Drawing for the job (mm, zero at the part's lowest x, y, z). A direction names the side the tool comes from. Round coordinates to 2 decimals unless told otherwise and drop trailing zeros. Write each loop counter-clockwise with the first axis right and the second up, starting at its lowest first coordinate (ties: lowest second). Pieces come first, ordered by that corner, then holes.
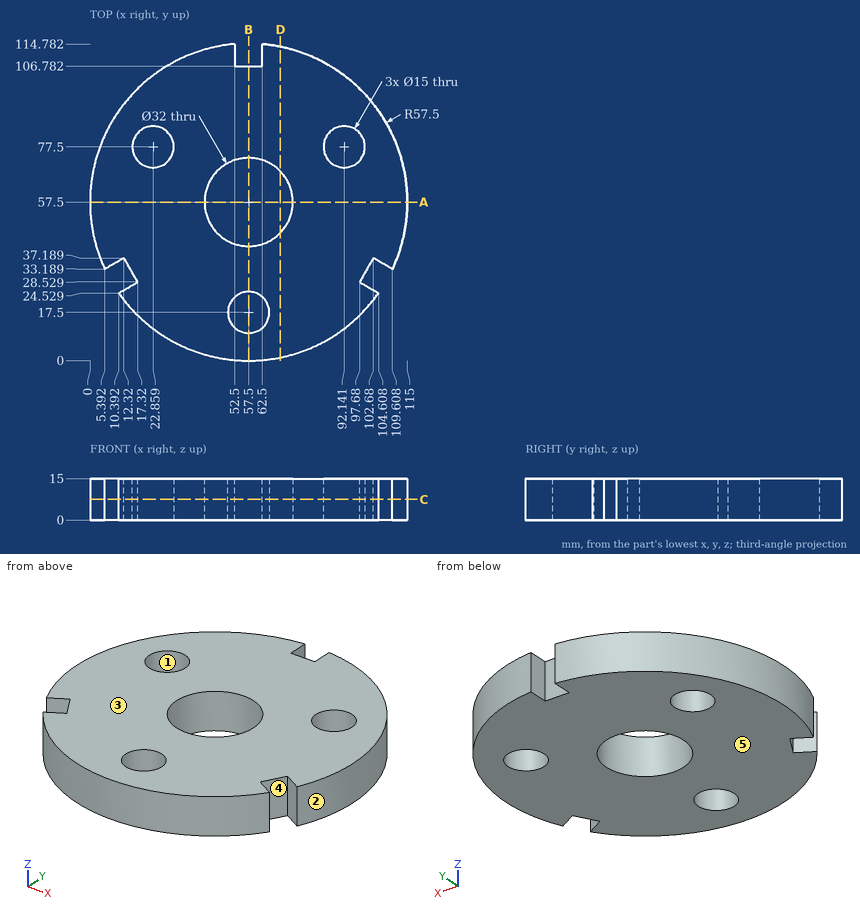
1) Which spindle directions (+Z, -Z, +X, -X, +Y, -Y) get a long thin tool onto all of the face, cutting with end or side? Do the marked faces 4 and 5. Say none if no direction does.
2) Wall check: probe 1 along Y at (x, z) = (57.5, 8); probe 2 along Y at (x, z) = (61, 11); probe 3 along X at (y, z) = (77, 1.25) (1 decimal). Give the ranges that are in metal, low to high.
3) Cut at C-C on z = 7.5. List the corners of the cut face in (x, y).
4) Flat gauge pins, fed straight in: pin 1 Ø2.5 at (y, z) = (109.5, 11) entering from +X; pin 2 Ø2.5 at (y, z) = (109.5, 4) entering from -X; pin 3 Ø4 at (y, z) = (22, 3) entering from -X. Where does each tip first touch, or does it go through?
5) Cut at B-B on x = 57.5. List the corners of the cut face in (y, z), and give its area (3 significant figures).
6) Pull direction Y, two halves, no side cores. Call the marked faces 1, 2 and 3: released by +Y, released by -Y, zero draft, split by the parting line, or undercut.
7) Cut at D-D on x = 69. List the corners of the cut face in (y, z) (1 decimal), and give its area (3 significant figures).
8) Cut at A-A on y = 57.5. List the corners of the cut face in (x, z).
Result sheet:
1. face 4: +Z, -Z
1. face 5: -Z, +X, -X, +Y, -Y
2. probe 1: y = 0 to 10, 25 to 41.5, 73.5 to 106.78
2. probe 2: y = 0.11 to 10.87, 24.13 to 41.89, 73.11 to 106.78
2. probe 3: x = 3.4 to 15.4, 30.3 to 84.7, 99.6 to 111.6
3. outline: (5.39, 33.19) - (12.32, 37.19) - (17.32, 28.53) - (10.39, 24.53) arc R57.5 ccw to (104.61, 24.53) - (97.68, 28.53) - (102.68, 37.19) - (109.61, 33.19) arc R57.5 ccw to (62.5, 114.78) - (62.5, 106.78) - (52.5, 106.78) - (52.5, 114.78) arc R57.5 ccw to start; hole circle Ø15 at (22.86, 77.5); hole circle Ø32 at (57.5, 57.5); hole circle Ø15 at (57.5, 17.5); hole circle Ø15 at (92.14, 77.5)
4. pin 1: stops at x = 84.53
4. pin 2: stops at x = 30.47
4. pin 3: stops at x = 10.77
5. outline: (0, 0) - (10, 0) - (10, 15) - (0, 15) - close; (25, 0) - (41.5, 0) - (41.5, 15) - (25, 15) - close; (73.5, 0) - (106.78, 0) - (106.78, 15) - (73.5, 15) - close
5. area: 897 mm2
6. face 1: undercut
6. face 2: split by the parting line
6. face 3: zero draft
7. outline: (1.2, 0) - (46.4, 0) - (46.4, 15) - (1.2, 15) - close; (68.6, 0) - (113.8, 0) - (113.8, 15) - (68.6, 15) - close
7. area: 1,360 mm2
8. outline: (0, 0) - (41.5, 0) - (41.5, 15) - (0, 15) - close; (73.5, 0) - (115, 0) - (115, 15) - (73.5, 15) - close
